from build123d import *

# Parameters (mm, degrees)
EXTRUDE_1_DEPTH = 260
FILLET_1_R      = 5


with BuildPart() as part:
    # 草图1 → 拉伸-薄壁1 (new body)
    with BuildSketch(Plane.XY):
        Polygon((40, 40), (0, 40), (0, -40), (40, -40), (40, -35), (5, -35), (5, 35), (40, 35), align=None)
    extrude(amount=EXTRUDE_1_DEPTH)

    # 圆角1
    fillet_1_edges = [part.edges().sort_by_distance(p)[0] for p in [
        (0, -40, 130),
        (0, 40, 130),
    ]]
    fillet(fillet_1_edges, radius=FILLET_1_R)


solid = part.part
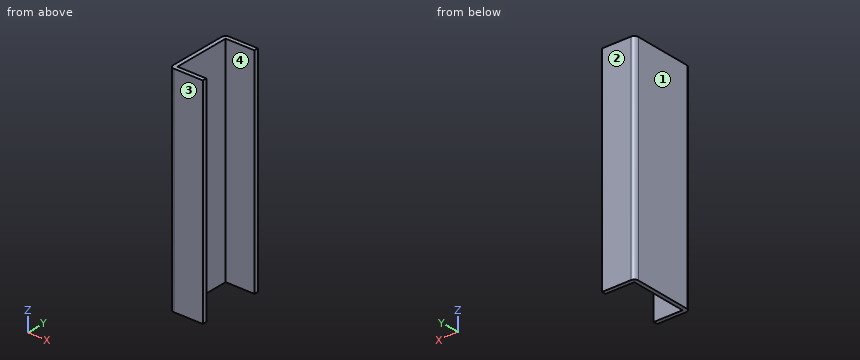
Geometry check sheet. Reference: the model listing, model coordinates, mm. Face numbers are marked on the shaded views. Round coordinates to 2 decimals unless told otherwise and drop trailing zeros. Order: outer loops, then holes, each group sorted by start corner. A loop starts at its lowest first (then second) coordinate and runs counter-clockwise, first axis right, second up. Notation, with made-up numbers: (26.25, -36.5) - (52.25, -36.5) arc R30 cw to (52.25, -14.5) - close; hole circle Ø1 at (42, 52). An arc over 180 degrees is marked (long way). One line per question, with ' | ' between items. Start each with the question number.
(1) Sectioned sample at C-C on y = -10.5. Record the cut outline in (x, z), and give its area (3 significant figures).
(2) Thickness scan on L1, parallel to Y at x = 26.5, z = 215.5; L2, parallel to X at y = 6, z = 247.5; L3, parallel to Y at x = 3, z = 139. Record the ranges inside material, lowest first. Write a range as [from, to].
(3) Sectioned sample at A-A on x = 8.5. Record the cut outline in (y, z).
(4) Release check for a two-part mould opening along Y. For the marked faces 1, 2, 3 and 4 record: released by +Y, released by -Y, zero draft, split by the parting line, or undercut.
(5) Sectioned sample at B-B on z = 116. Record the cut outline in (x, y), and give its area (3 significant figures).
(6) Depth check by flat-ended pin: pin 1 Ø5 at (y, z) = (0, 222.5) entering from +X. Enter the tip coordinate at first touch or a pass-through.
Conclusion:
1) outline: (0, 0) - (5, 0) - (5, 260) - (0, 260) - close | area: 1,300 mm2
2) L1: y = [-40, -35], [35, 40] | L2: x = [0, 5] | L3: y = [-39.58, 39.58]
3) outline: (-40, 0) - (-35, 0) - (-35, 260) - (-40, 260) - close; (35, 0) - (40, 0) - (40, 260) - (35, 260) - close
4) face 1: zero draft | face 2: released by +Y | face 3: released by -Y | face 4: undercut
5) outline: (0, -35) arc R5 ccw to (5, -40) - (40, -40) - (40, -35) - (5, -35) - (5, 35) - (40, 35) - (40, 40) - (5, 40) arc R5 ccw to (0, 35) - close | area: 739 mm2
6) pin 1: stops at x = 5
